The figure shows three views and two pictorial views of one solid part (mm, origin at its lowest corner). Answer the questions. A direction names the side the tool comes from. Round coordinates to 2 decimals unless told otherwise and drop trailing zeros. Write each loop counter-clockwise with the first axis right and the second up, starting at its lowest first coordinate (ties: lowest second). Pieces come first, ordered by that corner, then holes. Notation, with made-up numbers: M 20.5,69.25 L 32.5,69.25 A28 ccw 32.5,103.25 Z; hole C -40,-34.5 d4. An arc over 180 degrees is marked long. One line per item, written item: value. Start each with the question number.
Q1. Find section C-C (z = 7.25). Write down the section's boundary in (x, y), and give its area (3 significant figures).
Q2. Given pin 1 Ø2 at (x, z) = (30, 3.5) entering from +Y; pin 2 Ø3 at (y, z) = (38, 6) entering from +X; pin 3 Ø1 at (x, z) = (27.5, 7) entering from -Y, each flat-ended and moving along its own axis, determine where each tip first touches the part or whether it passes through.
Q3. Find section A-A (y = 25). Write down the section's boundary in (x, z).
Q4. A tool of negligible diameter and unlimited length cuts with its end or side. For the marked faces 4 and 5, from which of +Z, -Z, +X, -X, +Y, -Y can it reach the whole face along a straight path? Write none if from no direction.
Q5. Consider probe 1 along Y at (x, z) = (25, 4); probe 2 along Y at (x, z) = (16.5, 6) (1 decimal); probe 3 along X at (y, z) = (37.5, 3). Determine where each line is inside the solid, lowest interval first.
Q6. The mould has two halves that part along X. Classify the marked faces 1, 2 and 3: released by +X, released by -X, zero draft, split by the parting line, or undercut.
Q7. Find section D-D (x = 45). Write down the section's boundary in (y, z).
Q8. Find section B-B (x = 25). Write down the section's boundary in (y, z).
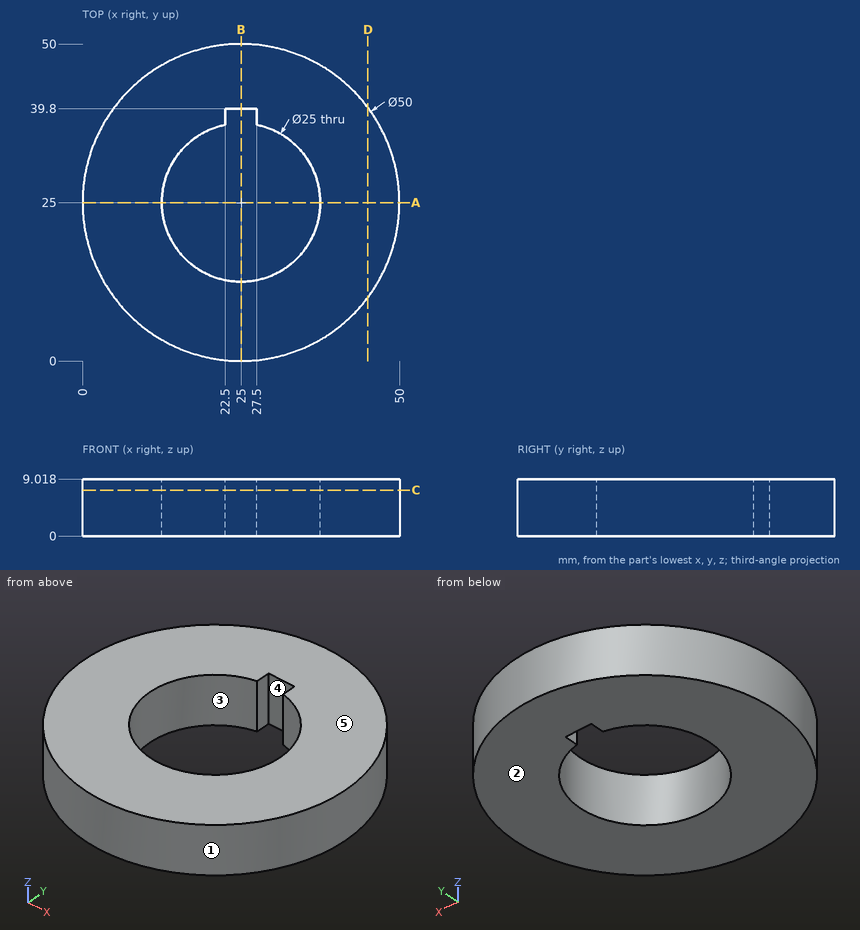
The answers:
1. outline: C 25,25 d50; hole M 22.5,37.25 A12.5 ccw long 27.5,37.25 L 27.5,39.8 L 22.5,39.8 Z
1. area: 1,460 mm2
2. pin 1: y = 49.68
2. pin 2: x = 47.2
2. pin 3: y = 0.08
3. outline: M 0,0 L 12.5,0 L 12.5,9.02 L 0,9.02 Z; M 37.5,0 L 50,0 L 50,9.02 L 37.5,9.02 Z
4. face 4: +Z, -Z
4. face 5: +Z, +X, -X, +Y, -Y
5. probe 1: 0 to 12.5, 39.8 to 50
5. probe 2: 1.5 to 15.8, 34.2 to 48.5
5. probe 3: 3.35 to 22.5, 27.5 to 46.65
6. face 1: split by the parting line
6. face 2: zero draft
6. face 3: undercut
7. outline: M 10,0 L 40,0 L 40,9.02 L 10,9.02 Z
8. outline: M 0,0 L 12.5,0 L 12.5,9.02 L 0,9.02 Z; M 39.8,0 L 50,0 L 50,9.02 L 39.8,9.02 Z
